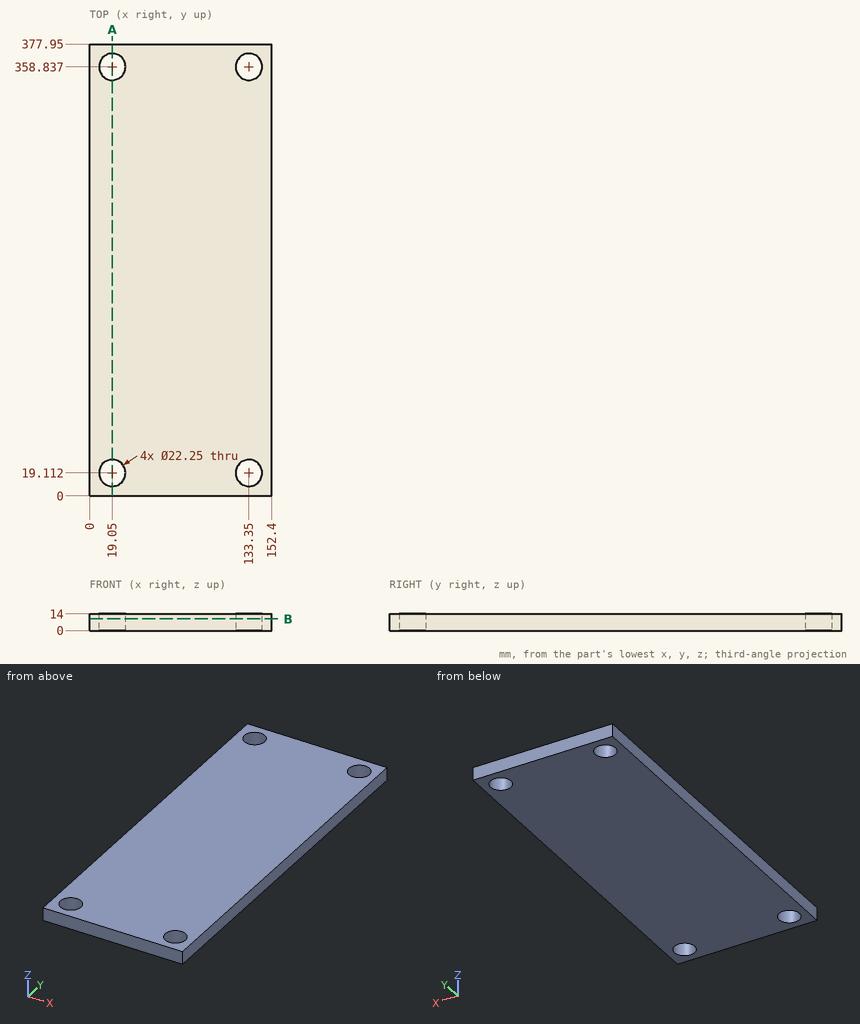
Study the drawing (mm; zero at the part's minimum x, y, z) and answer. Coordinates: 2 decimals unless noted, no trailing zeros. Loops run counter-clockwise (first coordinate to the right, second up) from the corner with the lowest first, then second, coordinate; pieces in that order, holes last. Notation, with made-up numbers: (84, 81.25) -> (132, 81.25) arc R8 ccw to (132, 90.25) -> close; hole circle Ø7 at (48, 34). An arc over 180 degrees is marked (long way). Write item = value, one per line. Start each with the question number.
1) The part is cut by section A-A, the plane x = 19.05. Determine the outline of the cut face in (y, z), plus the area to 3 significant figures.
2) Find the intervals of material crossed by L1, parallel to Y at x = 19.05, z = 10.25; L2, parallel to X at y = 359, z = 4; L3, parallel to X at y = 355.5, z = 12.5, in increasing order. Write a range as from..to.
3) The part is cut by section B-B, the plane z = 9.75. State how many separate pieces and enclosed holes the cut face has, plus the area to 3 significant figures.
4) Given P1, Ø13.5, axis at x = 133.35, y = 19.11, coming from the +Z side, flat-ended and moving along its own axis, determine where the tip first touches the part or whether it passes through.
Result:
q1.outline = (0, 0) -> (7.99, 0) -> (7.99, 14) -> (0, 14) -> close; (30.24, 0) -> (347.71, 0) -> (347.71, 14) -> (30.24, 14) -> close; (369.96, 0) -> (377.95, 0) -> (377.95, 14) -> (369.96, 14) -> close
q1.area = 4,670 mm²
q2.L1 = 0..7.99, 30.24..347.71, 369.96..377.95
q2.L2 = 0..7.93, 30.17..122.23, 144.47..152.4
q2.L3 = 0..8.44, 29.66..122.74, 143.96..152.4
q3.separate_pieces = 1
q3.enclosed_holes = 4
q3.area = 56,000 mm²
q4.P1 = through
